Work out the finished part from the listing and answer in its coordinate system (mm). A direction names the side the tool comes from. Coordinates: 2 decimals unless noted, no trailing zeros. Write each loop counter-clockwise with the first axis right and the second up, starting at its lowest first coordinate (ties: lowest second). Pieces come first, ordered by that corner, then holes. Notation, with made-up numbers: (18.5, 16.25) - (26.5, 16.25) arc R16 cw to (26.5, 21.25) - close; hole circle Ø4 at (32, 30). An arc over 180 degrees is marked (long way). Use one line per item in the form item = value. Start each with the question number.
Item 1: A cutting plane is placed at D-D (z = 10.75). Write down the section's boundary in (x, y).
Item 2: For faces 1 (the flat face through (0, 90, 0)), 2 (the cylindrical face through (-1.802, 7.605, -5.723)), 3 (the flat face through (8, 20, -2)), determine the directions among +Z, -Z, +X, -X, +Y, -Y from which every point of the face is accessible in a straight line to the end or side of a thin tool.
Item 3: Given pin 1 (10 mm diameter, centred on x = 9, z = 9, fed in from -Y); pin 2 (1.5 mm diameter, centred on x = -8.5, y = 65, fed in from -Z); pin 3 (12 mm diameter, centred on x = 1, y = 38, fed in from +Z); pin 4 (5 mm diameter, centred on y = 19.5, z = 9.5, fed in from +X), each flat-ended and moving along its own axis, determine where each tip first touches the part or whether it passes through.
Item 4: A cutting plane is placed at B-B (x = 0). Write down the section's boundary in (y, z), then the cut area to 3 significant figures.
Item 5: A cutting plane is placed at A-A (z = 0). Write down the section's boundary in (x, y), then the cut area to 3 significant figures.
Item 6: A cutting plane is placed at C-C (y = 61.5). Write down the section's boundary in (x, z).
Item 7: Consider probe 1 along Y at (x, z) = (-2.5, -8); probe 2 along X at (y, z) = (19.5, 10.5); probe 3 along X at (y, z) = (85.5, -4.75). Determine where each line is inside the solid, lowest interval first.
from build123d import *

# Parameters (mm, degrees)
COLLAR_FILLET_R2_R = 2


with BuildPart() as part:
    # Stud Profile Sketch → Stud Body Revolve (revolve)
    with BuildSketch(Plane.XY, mode=Mode.PRIVATE) as stud_body_revolve_sk:
        Polygon((0, 0), (6, 0), (6, 15), (12, 15), (12, 20), (6, 20), (6, 90), (0, 90), align=None)
    revolve(stud_body_revolve_sk.sketch.rotate(Axis((0, -19.657458564, 0), (0, 1, 0)), 90), axis=Axis((0, -19.657458564, 0), (0, 1, 0)))

    # Collar Fillet R2
    collar_fillet_r2_edges = [part.edges().sort_by_distance(p)[0] for p in [
        (0, 20, 6),
    ]]
    fillet(collar_fillet_r2_edges, radius=COLLAR_FILLET_R2_R)


solid = part.part
Answer:
q1.outline = (-5.33, 15) - (5.33, 15) - (5.33, 20) - (-5.33, 20) - close
q2.face_1 = +Z, -Z, +X, -X, +Y
q2.face_2 = -Y
q2.face_3 = +Y
q3.pin_1 = 15
q3.pin_2 = through
q3.pin_3 = 6
q3.pin_4 = 9.75
q4.outline = (0, -6) - (15, -6) - (15, -12) - (20, -12) - (20, -8) arc R2 cw to (22, -6) - (90, -6) - (90, 6) - (22, 6) arc R2 cw to (20, 8) - (20, 12) - (15, 12) - (15, 6) - (0, 6) - close
q4.area = 1,140 mm²
q5.outline = (-12, 15) - (-6, 15) - (-6, 0) - (6, 0) - (6, 15) - (12, 15) - (12, 20) - (8, 20) arc R2 cw to (6, 22) - (6, 90) - (-6, 90) - (-6, 22) arc R2 cw to (-8, 20) - (-12, 20) - close
q5.area = 1,140 mm²
q6.outline = circle Ø12 at (0, 0)
q7.probe_1 = 15 to 20
q7.probe_2 = -5.81 to 5.81
q7.probe_3 = -3.67 to 3.67
